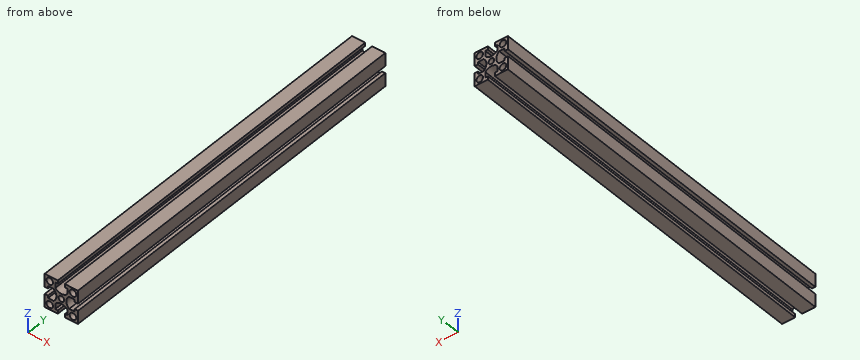
from build123d import *

# Parameters (mm, degrees)
SKETCH_3_R     = 4
SKETCH_3_R_2   = 3.4
EF4040_1_DEPTH = 455


with BuildPart() as part:
    # 草圖3 → 東野鋁型材 EF4040(1) (new body)
    with BuildSketch(Plane(origin=(0, 0, 0), x_dir=(-1, 0, 0), z_dir=(0, 1, 0))):
        with BuildLine():
            Line((-20, -20), (-4.2, -20))
            Line((-4.2, -20), (-4.2, -16))
            Line((-4.2, -16), (-7.25, -16))
            Line((-7.25, -16), (-7.25, -9.360985421))
            ThreePointArc((-7.25, -9.360985421), (0, -6), (7.25, -9.360985421))
            Line((7.25, -9.360985421), (7.25, -16))
            Line((7.25, -16), (4.2, -16))
            Line((4.2, -16), (4.2, -20))
            Line((4.2, -20), (20, -20))
            Line((20, -20), (20, -4.2))
            Line((20, -4.2), (16, -4.2))
            Line((16, -4.2), (16, -7.25))
            Line((16, -7.25), (9.360985421, -7.25))
            ThreePointArc((9.360985421, -7.25), (6, 0), (9.360985421, 7.25))
            Line((9.360985421, 7.25), (16, 7.25))
            Line((16, 7.25), (16, 4.2))
            Line((16, 4.2), (20, 4.2))
            Line((20, 4.2), (20, 20))
            Line((20, 20), (4.2, 20))
            Line((4.2, 20), (4.2, 16))
            Line((4.2, 16), (7.25, 16))
            Line((7.25, 16), (7.25, 9.360985421))
            ThreePointArc((7.25, 9.360985421), (0, 6), (-7.25, 9.360985421))
            Line((-7.25, 9.360985421), (-7.25, 16))
            Line((-7.25, 16), (-4.2, 16))
            Line((-4.2, 16), (-4.2, 20))
            Line((-4.2, 20), (-20, 20))
            Line((-20, 20), (-20, 4.2))
            Line((-20, 4.2), (-16, 4.2))
            Line((-16, 4.2), (-16, 7.25))
            Line((-16, 7.25), (-9.360985421, 7.25))
            ThreePointArc((-9.360985421, 7.25), (-6, 0), (-9.360985421, -7.25))
            Line((-9.360985421, -7.25), (-16, -7.25))
            Line((-16, -7.25), (-16, -4.2))
            Line((-16, -4.2), (-20, -4.2))
            Line((-20, -4.2), (-20, -20))
        make_face()
        with Locations((-13.999999649, -13.999999649)):
            Circle(SKETCH_3_R, mode=Mode.SUBTRACT)
        Circle(SKETCH_3_R_2, mode=Mode.SUBTRACT)
        with Locations((14.00000014, -13.999999158)):
            Circle(SKETCH_3_R, mode=Mode.SUBTRACT)
        with Locations((-13.999999649, 14.000000351)):
            Circle(SKETCH_3_R, mode=Mode.SUBTRACT)
        with Locations((13.999999158, 14.000000842)):
            Circle(SKETCH_3_R, mode=Mode.SUBTRACT)
    extrude(amount=EF4040_1_DEPTH)


solid = part.part
Design review of the part built by this model. Coordinates are the model's own, in mm. Coordinates: 2 decimals unless noted, no trailing zeros. Use one line per item in the form item = value.
(1) Clearance check with flat-ended pins moving along their axes: P1, Ø2, axis at x = -2.5, y = 242, coming from the -Z side; P2, Ø10.5, axis at x = -14, z = 14, coming from the +Y side; P3, Ø4, axis at x = 0, z = 0, coming from the +Y side. State where each tip first meets the part, or that it passes through.
Return value:
P1 = -6.67
P2 = 455
P3 = through
(2) For line 1 along Z through (x, y) = (14, 128.5); line 2 along X through (y, z) = (276, -13.5); line 3 along X through (y, z) = (396, -17), list the stretches that pass through material, from the lowest coordinate up. Write a range as from..to.
Return value:
line_1 = -20..-18, -10..-7.25, 7.25..10, 18..20
line_2 = -20..-17.97, -10.03..-7.25, 7.25..10.03, 17.97..20
line_3 = -20..-16.65, -11.35..-4.2, 4.2..11.35, 16.65..20
(3) Consider section A-A (y = 68.5). Give the number of separate pieces and of enclosed holes in the cut face, and give its area (3 significant figures).
Return value:
separate_pieces = 1
enclosed_holes = 5
area = 708 mm2
